Build history of the part. All positions in model axes, mm. Face numbers are marked on the shaded views. Round coordinates to 2 decimals unless told otherwise and drop trailing zeros. Order: outer loops, then holes, each group sorted by start corner. A loop starts at its lowest first (then second) coordinate and runs counter-clockwise, first axis right, second up. Notation, with made-up numbers: M 18.5,89 L 23.5,89 A18 ccw 23.5,98 Z; hole C -17.75,-9 d8. An arc over 180 degrees is marked long. Use CSV: the item, a comma, the result in double quotes.
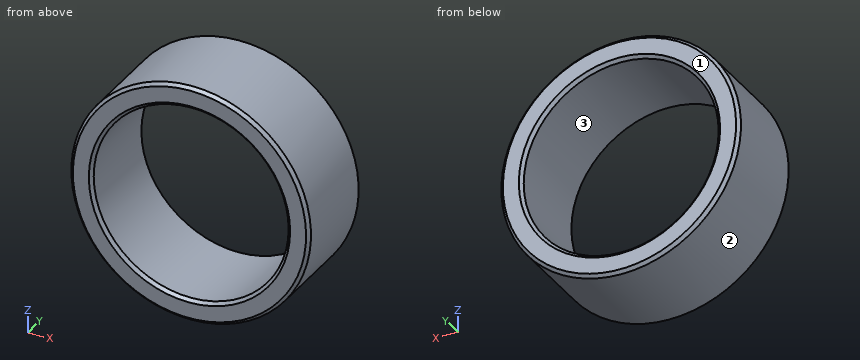
from build123d import *

# Parameters (mm, degrees)
SKETCH1_R           = 37.5
SKETCH1_R_2         = 30.5
BOSS_EXTRUDE1_DEPTH = 30
CHAMFER1_SIZE       = 1


with BuildPart() as part:
    # Sketch1 → Boss-Extrude1 (new body)
    with BuildSketch(Plane(origin=(0, 0, 0), x_dir=(1, 0, 0), z_dir=(0, 1, 0))):
        with Locations(Location((0, 0, 0), (0, 0, 270))):
            Circle(SKETCH1_R)
        with Locations(Location((0, 0, 0), (0, 0, 270))):
            Circle(SKETCH1_R_2, mode=Mode.SUBTRACT)
    extrude(amount=BOSS_EXTRUDE1_DEPTH)

    # Chamfer1
    chamfer1_edges = [part.edges().sort_by_distance(p)[0] for p in [
        (0, 0, -37.5),
        (0, 30, -37.5),
        (0, 0, -30.5),
        (0, 30, -30.5),
    ]]
    chamfer(chamfer1_edges, length=CHAMFER1_SIZE)


solid = part.part
(1) Cut at A-A, the plane z = 0. Give the cut face in (x, y).
Answer block:
outline,"M -37.5,1 L -36.5,0 L -31.5,0 L -30.5,1 L -30.5,29 L -31.5,30 L -36.5,30 L -37.5,29 Z; M 30.5,1 L 31.5,0 L 36.5,0 L 37.5,1 L 37.5,29 L 36.5,30 L 31.5,30 L 30.5,29 Z"
(2) Two-plate mould, pull along X, no slides. Class the marked faces 1, 2 and 3: released by +X, released by -X, zero draft, split by the parting line, or undercut.
Answer block:
face 1,"zero draft"
face 2,"split by the parting line"
face 3,"undercut"
(3) Wall check: line 1 (X direction, y = 10.5, z = 0); line 2 (X direction, y = 15.75, z = -5); line 3 (Z direction, x = 18.5, y = 20.5). Give the ranges that are in metal, low to high. Write a range as from..to.
Answer block:
line 1,"x = -37.5..-30.5, 30.5..37.5"
line 2,"x = -37.17..-30.09, 30.09..37.17"
line 3,"z = -32.62..-24.25, 24.25..32.62"
(4) Cut at C-C, the plane y = 19.25. Give the cut face in (x, z), and give its area (3 significant figures).
Answer block:
outline,"C 0,0 d75; hole C 0,0 d61"
area,"1,500 mm²"
(5) Drop flat-ended pins along their axis: pin 1 (3 mm diameter, centred on y = 17, z = 5, fed in from -X); pin 2 (10 mm diameter, centred on x = 27, y = 20.5, fed in from -Z); pin 3 (10 mm diameter, centred on x = 22, y = 18.5, fed in from -Z); pin 4 (1 mm diameter, centred on x = 27.5, z = 6, fed in from -Y). Give the stop position or say it passes through.
Answer block:
pin 1,"stops at x = -37.34"
pin 2,"stops at z = -30.37"
pin 3,"stops at z = -33.43"
pin 4,"passes through"
(6) Cut at B-B, the plane x = 0. Give the cut face in (y, z).
Answer block:
outline,"M 0,-36.5 L 1,-37.5 L 29,-37.5 L 30,-36.5 L 30,-31.5 L 29,-30.5 L 1,-30.5 L 0,-31.5 Z; M 0,31.5 L 1,30.5 L 29,30.5 L 30,31.5 L 30,36.5 L 29,37.5 L 1,37.5 L 0,36.5 Z"
